For this review, take the finished solid that the model builds, in its own axes (mm). Face numbers are marked on the shaded views. A direction names the side the tool comes from. Round coordinates to 2 decimals unless told otherwise and drop trailing zeros. Order: outer loops, then holes, each group sorted by start corner. A loop starts at its lowest first (then second) coordinate and runs counter-clockwise, first axis right, second up. Notation, with made-up numbers: M -33,50 L -22,50 A9 cw -22,66 Z; hole C 1.5,86.25 d8. An arc over 180 degrees is marked long. Answer as a JSON object with one key per item and string values.
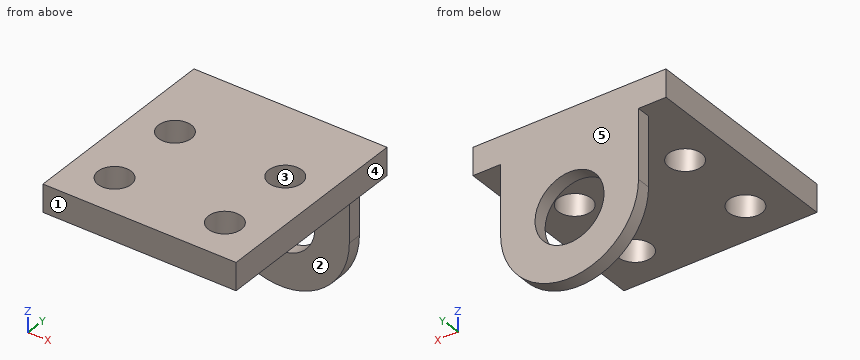
from build123d import *

# Parameters (mm, degrees)
SKETCH_1_W          = 70
SKETCH_1_H          = 70
SKETCH_1_R          = 6
EXTRUDE_1_DEPTH     = 10
SKETCH_2_W          = 70
SKETCH_2_H          = 5
EXTRUDE_2_DEPTH     = 60
SKETCH_4_R          = 12.5
CUT_EXTRUDE_1_DEPTH = 10


with BuildPart() as part:
    # 草图1 → 凸台-拉伸1 (new body)
    with BuildSketch(Plane.XY):
        with Locations((20, 20)):
            Rectangle(SKETCH_1_W, SKETCH_1_H)
        Circle(SKETCH_1_R, mode=Mode.SUBTRACT)
        with Locations((0, 30)):
            Circle(SKETCH_1_R, mode=Mode.SUBTRACT)
        with Locations((40, 30)):
            Circle(SKETCH_1_R, mode=Mode.SUBTRACT)
        with Locations((40, 0)):
            Circle(SKETCH_1_R, mode=Mode.SUBTRACT)
    extrude(amount=EXTRUDE_1_DEPTH)

    # 草图2 → 凸台-拉伸2 (add)
    with BuildSketch(Plane.XY.offset(10)):
        with Locations((20, 57.5)):
            Rectangle(SKETCH_2_W, SKETCH_2_H)
    extrude(amount=-EXTRUDE_2_DEPTH)

    # 草图4 → 切除-拉伸1 (cut)
    with BuildSketch(Plane(origin=(0, 60, 0), x_dir=(1, 0, 0), z_dir=(0, 1, 0))):
        with Locations(Location((20, 25, 0), (0, 0, 270))):
            Circle(SKETCH_4_R)
        with BuildLine():
            Line((-5, 25), (-5, 0))
            Line((-5, 0), (-23.267990544, 0))
            Line((-23.267990544, 0), (-23.267990544, 53.705684911))
            Line((-23.267990544, 53.705684911), (55, 53.705684911))
            Line((55, 53.705684911), (55, 0))
            Line((55, 0), (45, 0))
            Line((45, 0), (45, 25))
            ThreePointArc((45, 25), (20, 50), (-5, 25))
        make_face()
    extrude(amount=-CUT_EXTRUDE_1_DEPTH, mode=Mode.SUBTRACT)


solid = part.part
1) Machinability: for the marked faces 1 and 2, which of the approach directions +Z, -Z, +X, -X, +Y, -Y give a long, thin tool a straight path to every point of the face, cutting with its end or side? Answer none if there is none.
Geometry check:
{"face 1": "+Z, -Z, +X, -X, -Y", "face 2": "-Z, +X, -X, -Y"}
2) Insertion check: P1, Ø14, axis at x = 0, y = 0, coming from the -Z side; P2, Ø11, axis at x = 40, y = 30, coming from the +Z side; P3, Ø5, axis at x = 30.5, z = -6, coming from the -Y side; P4, Ø5.5, axis at y = 57.5, z = -14, coming from the -X side. Each pin has a flat end and moves straight along its axis. Give the tip position at first contact, or say it passes through.
Geometry check:
{"P1": "stops at z = 0", "P2": "passes through", "P3": "stops at y = 55", "P4": "stops at x = -5"}
3) Mouldability with a two-part tool opening along X and no side actions: class the marked faces 3, 4 and 5 as +X half, -X half, draft (parallel to the pull), parting line (faces both ways), or undercut.
Geometry check:
{"face 3": "undercut", "face 4": "+X half", "face 5": "draft"}
4) Add section C-C on z = -17. State the section outline as (x, y) points.
Geometry check:
{"outline": "M -5,55 L 10.4,55 L 10.4,60 L -5,60 Z; M 29.6,55 L 45,55 L 45,60 L 29.6,60 Z"}
5) Add section A-A on x = 40. State the section outline as (y, z) points.
Geometry check:
{"outline": "M -15,0 L -6,0 L -6,10 L -15,10 Z; M 6,0 L 24,0 L 24,10 L 6,10 Z; M 36,0 L 55,0 L 55,-40 L 60,-40 L 60,10 L 36,10 Z"}
6) For L1, parallel to Y at x = 40, z = 7.5; L2, parallel to X at y = 58.4, z = -25; L3, parallel to Z at x = 28, y = 48, list the stretches that pass through material, from the lowest coordinate up.
Geometry check:
{"L1": "y = -15 to -6, 6 to 24, 36 to 60", "L2": "x = -5 to 7.5, 32.5 to 45", "L3": "z = 0 to 10"}
7) Add section B-B on y = 30. State the section outline as (x, z) points.
Geometry check:
{"outline": "M -15,0 L -6,0 L -6,10 L -15,10 Z; M 6,0 L 34,0 L 34,10 L 6,10 Z; M 46,0 L 55,0 L 55,10 L 46,10 Z"}
8) Add section D-D on x = 20. State the section outline as (y, z) points, and give its area (3 significant figures).
Geometry check:
{"outline": "M -15,0 L 55,0 L 55,-12.5 L 60,-12.5 L 60,10 L -15,10 Z; M 55,-50 L 60,-50 L 60,-37.5 L 55,-37.5 Z", "area": "875 mm²"}
